The listing builds one solid part. Answer for the finished solid, in the listing's coordinates (mm). Give positions to 0.01 mm unless a question says otherwise; leave off trailing zeros. Write each loop counter-clockwise with the first axis right and the second up, starting at its lowest first coordinate (ties: lowest second). Pieces come first, ordered by that corner, then holes. Notation, with made-up numbers: (24, 35) - (42, 35) arc R16 ccw to (42, 44) - close; hole circle Ø9 at (80.5, -16). An arc over 180 degrees is marked (long way). Use a Markdown table: item, result. Add a question column.
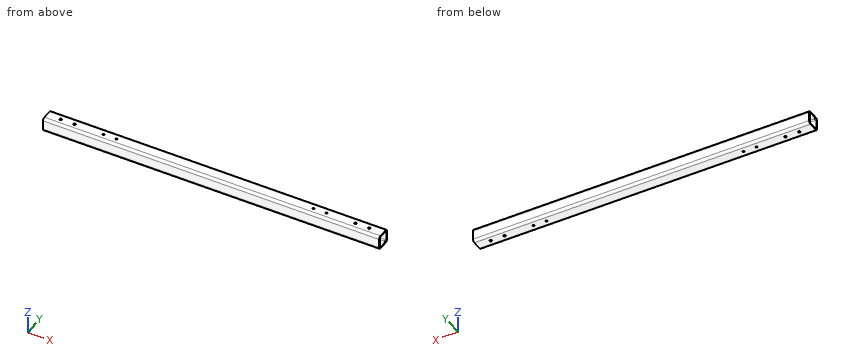
from build123d import *

# Parameters (mm, degrees)
MEMBER_1_DEPTH     = 730
HOLE_WIZARD_M5_1_D = 4.2
HOLE_WIZARD_M6_1_D = 5


with BuildPart() as part:
    # Sketch1 → Member 1 (new body)
    with BuildSketch(Plane(origin=(0, 0, 0), x_dir=(0, 0, -1), z_dir=(1, 0, 0))):
        with BuildLine():
            Line((-9.8, -15), (9.8, -15))
            ThreePointArc((9.8, -15), (13.476955262, -13.476955262), (15, -9.8))
            Line((15, -9.8), (15, 9.8))
            ThreePointArc((15, 9.8), (13.476955262, 13.476955262), (9.8, 15))
            Line((9.8, 15), (-9.8, 15))
            ThreePointArc((-9.8, 15), (-13.476955262, 13.476955262), (-15, 9.8))
            Line((-15, 9.8), (-15, -9.8))
            ThreePointArc((-15, -9.8), (-13.476955262, -13.476955262), (-9.8, -15))
        make_face()
        with BuildLine():
            Line((-9.8, -12.4), (9.8, -12.4))
            ThreePointArc((9.8, -12.4), (11.638477631, -11.638477631), (12.4, -9.8))
            Line((12.4, -9.8), (12.4, 9.8))
            ThreePointArc((12.4, 9.8), (11.638477631, 11.638477631), (9.8, 12.4))
            Line((9.8, 12.4), (-9.8, 12.4))
            ThreePointArc((-9.8, 12.4), (-11.638477631, 11.638477631), (-12.4, 9.8))
            Line((-12.4, 9.8), (-12.4, -9.8))
            ThreePointArc((-12.4, -9.8), (-11.638477631, -11.638477631), (-9.8, -12.4))
        make_face(mode=Mode.SUBTRACT)
    extrude(amount=MEMBER_1_DEPTH)

    # M5 螺纹孔1 (through all)
    with Locations(Plane.XY.offset(15)):
        with Locations((123.2, 0), (151.2, 0), (606.8, 0), (578.8, 0)):
            Hole(HOLE_WIZARD_M5_1_D / 2)

    # M6 螺纹孔1 (through all)
    with Locations(Plane.XY.offset(15)):
        with Locations((30, 0), (60, 0), (700, 0), (670, 0)):
            Hole(HOLE_WIZARD_M6_1_D / 2)


solid = part.part
1. Consider L1, parallel to Y at x = 223.5, z = 7.5; L2, parallel to Y at x = 578.8, z = -13.05. Determine where each line is inside the solid, lowest interval first. Write a range as [from, to].
2. The part is cut by section B-B (x = 84.5). Give the vertices of the cut face in (y, z).
3. The part is cut by section A-A (z = 0.75). Give the vertices of the cut face in (x, y).
Check values:
| question | item | result |
|---|---|---|
| 1 | L1 | y = [-15, -12.4], [12.4, 15] |
| 1 | L2 | y = [-13.86, -2.1], [2.1, 13.86] |
| 2 | outline | (-15, -9.8) arc R5.2 ccw to (-9.8, -15) - (9.8, -15) arc R5.2 ccw to (15, -9.8) - (15, 9.8) arc R5.2 ccw to (9.8, 15) - (-9.8, 15) arc R5.2 ccw to (-15, 9.8) - close; hole (-12.4, -9.8) arc R2.6 ccw to (-9.8, -12.4) - (9.8, -12.4) arc R2.6 ccw to (12.4, -9.8) - (12.4, 9.8) arc R2.6 ccw to (9.8, 12.4) - (-9.8, 12.4) arc R2.6 ccw to (-12.4, 9.8) - close |
| 3 | outline | (0, -15) - (730, -15) - (730, -12.4) - (0, -12.4) - close; (0, 12.4) - (730, 12.4) - (730, 15) - (0, 15) - close |
